from build123d import *

# Parameters (mm, degrees)
SKETCH1_W           = 40
SKETCH1_H           = 40
SKETCH1_W_2         = 36
SKETCH1_H_2         = 36
BOSS_EXTRUDE1_DEPTH = 860
FILLET1_R           = 2
FILLET2_R           = 4


with BuildPart() as part:
    # Sketch1 → Boss-Extrude1 (new body)
    with BuildSketch(Plane.XY):
        Rectangle(SKETCH1_W, SKETCH1_H)
        Rectangle(SKETCH1_W_2, SKETCH1_H_2, mode=Mode.SUBTRACT)
    extrude(amount=BOSS_EXTRUDE1_DEPTH)

    # Fillet1
    fillet1_edges = [part.edges().sort_by_distance(p)[0] for p in [
        (18, -18, 430),
        (18, 18, 430),
        (-18, 18, 430),
        (-18, -18, 430),
    ]]
    fillet(fillet1_edges, radius=FILLET1_R)

    # Fillet2
    fillet2_edges = [part.edges().sort_by_distance(p)[0] for p in [
        (20, -20, 430),
        (-20, -20, 430),
        (-20, 20, 430),
        (20, 20, 430),
    ]]
    fillet(fillet2_edges, radius=FILLET2_R)


solid = part.part
Source: CAD feature listing. Evaluate the final solid. Frame: model axes, mm. A direction names the side the tool comes from. Give positions to 0.01 mm unless a question says otherwise; leave off trailing zeros. Order: outer loops, then holes, each group sorted by start corner. A loop starts at its lowest first (then second) coordinate and runs counter-clockwise, first axis right, second up. Notation, with made-up numbers: (28.25, 82) -> (56.25, 82) arc R14 ccw to (56.25, 92) -> close; hole circle Ø2 at (17.5, 51). An arc over 180 degrees is marked (long way). Write item = value, one per line.
Q1. Pull-direction query (Y, two-part tool) for faces 1 (the face through (0, 20, 424)), 2 (the face through (-2, -19, 0)), 3 (the face through (18, 0, 424)); classes: released by +Y, released by -Y, zero draft, split by the parting line, or undercut.
Data:
face_1 = released by +Y
face_2 = zero draft
face_3 = undercut
Q2. Material intervals for line 1 (Y direction, x = 5, z = 159.5); line 2 (Y direction, x = 17.5, z = 660), sorted ascending. Write a range as from..to.
Data:
line_1 = -20..-18, 18..20
line_2 = -19.71..-17.32, 17.32..19.71
Q3. Cut plane B-B, the plane z = 786. Output: boundary loops of the cut face in (x, y).
Data:
outline = (-20, -16) arc R4 ccw to (-16, -20) -> (16, -20) arc R4 ccw to (20, -16) -> (20, 16) arc R4 ccw to (16, 20) -> (-16, 20) arc R4 ccw to (-20, 16) -> close; hole (-18, -16) arc R2 ccw to (-16, -18) -> (16, -18) arc R2 ccw to (18, -16) -> (18, 16) arc R2 ccw to (16, 18) -> (-16, 18) arc R2 ccw to (-18, 16) -> close
Q4. Pin query (flat end, axial travel): pin 1 (3 mm diameter, centred on x = -3, y = 15.5, fed in from +Z). Return the tip coordinate at first contact, or that it passes through.
Data:
pin_1 = through
Q5. Set-up query: faces 4 (the face through (-2, -19, 860)), 5 (the face through (-18, 0, 424)). Return all of +Z, -Z, +X, -X, +Y, -Y with unobstructed straight access to the full face (end or side cutting, diameter ignored); none if empty.
Data:
face_4 = +Z, +X, -X, +Y, -Y
face_5 = +Z, -Z
Q6. Cut plane A-A, the plane y = -8. Output: boundary loops of the cut face in (x, z), and give its area (3 significant figures).
Data:
outline = (-20, 0) -> (-18, 0) -> (-18, 860) -> (-20, 860) -> close; (18, 0) -> (20, 0) -> (20, 860) -> (18, 860) -> close
area = 3,440 mm^2
